```python
from build123d import *

# Parameters (mm, degrees)
EXTRUDE_1_DEPTH      = 125
EXTRUDE_2_DEPTH      = 20
EXTRUDE_2_DEPTH_BACK = 145
SKETCH_2_R           = 9.5
SKETCH_2_R_2         = 8


with BuildPart() as part:
    # 草图1 → 凸台-拉伸1 (new body)
    with BuildSketch(Plane.XY):
        with BuildLine():
            Line((-4, 10.246950766), (-4, 8.61684397))
            ThreePointArc((-4, 8.61684397), (-6.717514421, 6.717514421), (-8.61684397, 4))
            Line((-8.61684397, 4), (-10.246950766, 4))
            ThreePointArc((-10.246950766, 4), (-11, 0), (-10.246950766, -4))
            Line((-10.246950766, -4), (-8.61684397, -4))
            ThreePointArc((-8.61684397, -4), (-6.717514421, -6.717514421), (-4, -8.61684397))
            Line((-4, -8.61684397), (-4, -10.246950766))
            ThreePointArc((-4, -10.246950766), (0, -11), (4, -10.246950766))
            Line((4, -10.246950766), (4, -8.61684397))
            ThreePointArc((4, -8.61684397), (6.717514421, -6.717514421), (8.61684397, -4))
            Line((8.61684397, -4), (10.246950766, -4))
            ThreePointArc((10.246950766, -4), (11, 0), (10.246950766, 4))
            Line((10.246950766, 4), (8.61684397, 4))
            ThreePointArc((8.61684397, 4), (6.717514421, 6.717514421), (4, 8.61684397))
            Line((4, 8.61684397), (4, 10.246950766))
            ThreePointArc((4, 10.246950766), (0, 11), (-4, 10.246950766))
        make_face()
        with BuildLine():
            Line((-2.5, 9.16515139), (-2.5, 7.599342077))
            ThreePointArc((-2.5, 7.599342077), (-5.656854249, 5.656854249), (-7.599342077, 2.5))
            Line((-7.599342077, 2.5), (-9.16515139, 2.5))
            ThreePointArc((-9.16515139, 2.5), (-9.5, 0), (-9.16515139, -2.5))
            Line((-9.16515139, -2.5), (-7.599342077, -2.5))
            ThreePointArc((-7.599342077, -2.5), (-5.656854249, -5.656854249), (-2.5, -7.599342077))
            Line((-2.5, -7.599342077), (-2.5, -9.16515139))
            ThreePointArc((-2.5, -9.16515139), (0, -9.5), (2.5, -9.16515139))
            Line((2.5, -9.16515139), (2.5, -7.599342077))
            ThreePointArc((2.5, -7.599342077), (5.656854249, -5.656854249), (7.599342077, -2.5))
            Line((7.599342077, -2.5), (9.16515139, -2.5))
            ThreePointArc((9.16515139, -2.5), (9.5, 0), (9.16515139, 2.5))
            Line((9.16515139, 2.5), (7.599342077, 2.5))
            ThreePointArc((7.599342077, 2.5), (5.656854249, 5.656854249), (2.5, 7.599342077))
            Line((2.5, 7.599342077), (2.5, 9.16515139))
            ThreePointArc((2.5, 9.16515139), (0, 9.5), (-2.5, 9.16515139))
        make_face(mode=Mode.SUBTRACT)
    extrude(amount=EXTRUDE_1_DEPTH)

    # 草图2 → 凸台-拉伸2 (add, two sides: drawn at the far end of the back side and taken through both)
    with BuildSketch(Plane.XY.offset(125).offset(-EXTRUDE_2_DEPTH_BACK)):
        Circle(SKETCH_2_R)
        Circle(SKETCH_2_R_2, mode=Mode.SUBTRACT)
    extrude(amount=EXTRUDE_2_DEPTH + EXTRUDE_2_DEPTH_BACK)


solid = part.part
```
The listing builds one solid part. Answer for the finished solid, in the listing's coordinates (mm). Round coordinates to 2 decimals unless told otherwise and drop trailing zeros. Loops run counter-clockwise (first coordinate to the right, second up) from the corner with the lowest first, then second, coordinate; pieces in that order, holes last.
Q1. Section A-A, the plane x = 0 is taken. Determine the outline of the cut face in (y, z), then the cut area to 3 significant figures.
Q2. Given pin 1 Ø2.5 at (x, y) = (0.5, 10) entering from -Z; pin 2 Ø0.5 at (y, z) = (-9.5, 87.5) entering from +X; pin 3 Ø1.3 at (x, z) = (9.5, 48.5) entering from -Y; pin 4 Ø1.9 at (x, y) = (0, -10.5) entering from +Z, each flat-ended and moving along its own axis, determine where each tip first touches the part or whether it passes through.
Q3. For a pull along Y with two mould halves and no side action, classify faces 1 (the face through (0, 11, 62)), 2 (the face through (-1.73, -7.81, 61.34)), 3 (the face through (-4.3, -7, -20)) as released by +Y, released by -Y, zero draft, split by the parting line, or undercut.
Q4. Find the intervals of material crossed by line 1 (Y direction, x = 0, z = 57); line 2 (Z direction, x = 9.5, y = -3.75); line 3 (Y direction, x = -5.75, z = 71.5), in increasing order.
Q5. Section D-D, the plane y = -6.5 is taken. Determine the outline of the cut face in (x, z).
Q6. Section C-C, the plane z = 119 is taken. Determine the outline of the cut face in (x, y), then the cut area to 3 significant figures.
Completed:
1. outline: (-11, 0) - (-9.5, 0) - (-9.5, -20) - (-8, -20) - (-8, 145) - (-9.5, 145) - (-9.5, 125) - (-11, 125) - close; (8, -20) - (9.5, -20) - (9.5, 0) - (11, 0) - (11, 125) - (9.5, 125) - (9.5, 145) - (8, 145) - close
1. area: 870 mm2
2. pin 1: stops at z = -20
2. pin 2: stops at x = 4
2. pin 3: stops at y = -4
2. pin 4: stops at z = 125
3. face 1: released by +Y
3. face 2: undercut
3. face 3: zero draft
4. line 1: y = -11 to -8, 8 to 11
4. line 2: z = 0 to 125
4. line 3: y = -7.56 to -5.56, 5.56 to 7.56
5. outline: (-6.93, -20) - (-4.66, -20) - (-4.66, 145) - (-6.93, 145) - close; (4.66, -20) - (6.93, -20) - (6.93, 145) - (4.66, 145) - close
6. outline: (-10.25, -4) - (-8.62, -4) arc R9.5 ccw to (-4, -8.62) - (-4, -10.25) arc R11 ccw to (4, -10.25) - (4, -8.62) arc R9.5 ccw to (8.62, -4) - (10.25, -4) arc R11 ccw to (10.25, 4) - (8.62, 4) arc R9.5 ccw to (4, 8.62) - (4, 10.25) arc R11 ccw to (-4, 10.25) - (-4, 8.62) arc R9.5 ccw to (-8.62, 4) - (-10.25, 4) arc R11 ccw to start; hole circle Ø16 at (0, 0)
6. area: 132 mm2
